```python
from build123d import *

# Parameters (mm, degrees)
SKETCH_1_W          = 50
SKETCH_1_H          = 82.5
EXTRUDE_1_DEPTH     = 20
SKETCH_2_R          = 7
CUT_EXTRUDE_1_DEPTH = 53.216496436
SKETCH_3_W          = 10
SKETCH_3_H          = 70.5
CUT_EXTRUDE_2_DEPTH = 53.216496436


with BuildPart() as part:
    # 草图1 → 凸台-拉伸1 (new body)
    with BuildSketch(Plane.XY):
        Rectangle(SKETCH_1_W, SKETCH_1_H)
    extrude(amount=EXTRUDE_1_DEPTH)

    # 草图2 → 切除-拉伸1 (cut, through all)
    with BuildSketch(Plane.XY.offset(20)):
        with Locations((0, 23.75)):
            Circle(SKETCH_2_R)
    extrude(amount=-CUT_EXTRUDE_1_DEPTH, mode=Mode.SUBTRACT)

    # 草图3 → 切除-拉伸2 (cut, through all)
    with BuildSketch(Plane.XY.offset(20)):
        with Locations((-20, 6)):
            Rectangle(SKETCH_3_W, SKETCH_3_H)
        with Locations((20, 6)):
            Rectangle(SKETCH_3_W, SKETCH_3_H)
    extrude(amount=-CUT_EXTRUDE_2_DEPTH, mode=Mode.SUBTRACT)


solid = part.part
```
Could you check a few things on this model? Use its own coordinates, in mm. A direction names the side the tool comes from. Coordinates: 2 decimals unless noted, no trailing zeros. Loops run counter-clockwise (first coordinate to the right, second up) from the corner with the lowest first, then second, coordinate; pieces in that order, holes last.
1) Imagine slicing it at B-B (z = 5). List the corners of the cut face in (x, y) for me, and give its area (3 significant figures).
Reported:
outline: (-25, -41.25) - (25, -41.25) - (25, -29.25) - (15, -29.25) - (15, 41.25) - (-15, 41.25) - (-15, -29.25) - (-25, -29.25) - close; hole circle Ø14 at (0, 23.75)
area: 2,560 mm2
2) Imagine slicing it at C-C (x = 0). List the corners of the cut face in (y, z) for me, and give its area (3 significant figures).
Reported:
outline: (-41.25, 0) - (16.75, 0) - (16.75, 20) - (-41.25, 20) - close; (30.75, 0) - (41.25, 0) - (41.25, 20) - (30.75, 20) - close
area: 1,370 mm2
3) Which directions (+Z, -Z, +X, -X, +Y, -Y) give clear straight access to the entire face, cutting with the end or side of a thin tool? Please do faces 1 (the face through (-20, -29.25, 10)), 2 (the face through (15, 6, 10)), 3 (the face through (-1.517, 16.916, 10.14)).
Reported:
face 1: +Z, -Z, -X, +Y
face 2: +Z, -Z, +X, +Y
face 3: +Z, -Z
4) Will these pins go through, and if not, where does the flat tip stop? pin 1 Ø1.5 at (y, z) = (25, 8) entering from -X; pin 2 Ø5 at (x, z) = (21, 14) entering from +Y; pin 3 Ø3 at (x, y) = (17.5, 29.5) entering from -Z; pin 4 Ø6 at (y, z) = (-8, 13) entering from +X.
Reported:
pin 1: stops at x = -15
pin 2: stops at y = -29.25
pin 3: passes through
pin 4: stops at x = 15
5) Imagine slicing it at D-D (y = 13). List the corners of the cut face in (x, z) for me.
Reported:
outline: (-15, 0) - (15, 0) - (15, 20) - (-15, 20) - close
6) Imagine slicing it at A-A (y = 23.75). List the corners of the cut face in (x, z) for me.
Reported:
outline: (-15, 0) - (-7, 0) - (-7, 20) - (-15, 20) - close; (7, 0) - (15, 0) - (15, 20) - (7, 20) - close
7) Please list where these lines run through material, in increasing order: line 1 along Y through (x, z) = (0, 9.25); line 2 along X through (y, z) = (2, 2.25); line 3 along Y through (x, z) = (-22.5, 17.75).
Reported:
line 1: y = -41.25 to 16.75, 30.75 to 41.25
line 2: x = -15 to 15
line 3: y = -41.25 to -29.25
